Design review of the part built by this model. Coordinates are the model's own, in mm. A direction names the side the tool comes from. Give positions to 0.01 mm unless a question says otherwise; leave off trailing zeros. Order: outer loops, then holes, each group sorted by start corner. A loop starts at its lowest first (then second) coordinate and runs counter-clockwise, first axis right, second up. Notation, with made-up numbers: (86, -1.75) -> (129, -1.75) arc R20 cw to (129, 2.25) -> close; hole circle Ø10 at (40.25, 52.5). An arc over 180 degrees is marked (long way). Use a Markdown table: item, result. Add a question column.
```python
from build123d import *

# Parameters (mm, degrees)
BASE_BLOCK_DEPTH         = 50
POCKET_PROFILE_W         = 20
POCKET_PROFILE_H         = 35
RECTANGULAR_POCKET_DEPTH = 40
SLOT_PROFILE_W           = 30
SLOT_PROFILE_H           = 5
RECTANGULAR_SLOT_DEPTH   = 87.890735985


with BuildPart() as part:
    # Base Block Profile → Base Block (new body)
    with BuildSketch(Plane.XY):
        Polygon((0, 0), (80, 0), (80, 25), (100, 25), (100, 45), (55, 45), (55, 35), (0, 35), align=None)
    extrude(amount=BASE_BLOCK_DEPTH)

    # Pocket Profile → Rectangular Pocket (cut)
    with BuildSketch(Plane.ZY):
        with Locations((25, 17.5)):
            Rectangle(POCKET_PROFILE_W, POCKET_PROFILE_H)
    extrude(amount=-RECTANGULAR_POCKET_DEPTH, mode=Mode.SUBTRACT)

    # Slot Profile → Rectangular Slot (cut, through all)
    with BuildSketch(Plane.ZY.offset(-55)):
        with Locations((25, 42.5)):
            Rectangle(SLOT_PROFILE_W, SLOT_PROFILE_H)
    extrude(amount=-RECTANGULAR_SLOT_DEPTH, mode=Mode.SUBTRACT)


solid = part.part
```
1) Add section D-D (y = 33.5). Give the boundary of the cut face in (x, z).
2) The part is to be moulded in two halves that separate along Z. For faces 1 (the flat face through (55, 39, 25)), 2 (the flat face through (49, 23, 50)), 3 (the flat face through (20, 17, 15)), 4 (the flat face through (77, 42, 10)), say which applies: +Z half, -Z half, draft (parallel to the pull), parting line (faces both ways), or undercut.
3) Add section B-B (y = 41). Give the boundary of the cut face in (x, z), then the cut area to 3 significant figures.
4) Add section C-C (x = 77.5). Give the boundary of the cut face in (y, z).
5) For L1, parallel to Z at x = 89, y = 41; L2, parallel to Z at x = 9, y = 33.5; L3, parallel to X at y = 15, z = 46, list the stretches that pass through material, from the lowest coordinate up. Write a range as [from, to].
6) Machinability: for faces 5 (the flat face through (90, 25, 25)), 6 (the flat face through (28, 35, 36)), 7 (the flat face through (20, 17, 35)), which of the approach directions +Z, -Z, +X, -X, +Y, -Y give a long, thin tool a straight path to every point of the face, cutting with its end or side? Answer none if there is none.
7) Add section A-A (x = 11.5). Give the boundary of the cut face in (y, z), then the cut area to 3 significant figures.
8) Insertion check: pin 1 (12.5 mm diameter, centred on y = 13.5, z = 24, fed in from +X); pin 2 (2 mm diameter, centred on x = 46.5, z = 32, fed in from +Y); pin 3 (6 mm diameter, centred on x = 86.5, z = 29.5, fed in from -Y). Each pin has a flat end and moves straight along its axis. Give the tip position at first contact, or say it passes through.
Worked answers:
| question | item | result |
|---|---|---|
| 1 | outline | (0, 0) -> (100, 0) -> (100, 50) -> (0, 50) -> (0, 35) -> (40, 35) -> (40, 15) -> (0, 15) -> close |
| 2 | face 1 | draft |
| 2 | face 2 | +Z half |
| 2 | face 3 | undercut |
| 2 | face 4 | undercut |
| 3 | outline | (55, 0) -> (100, 0) -> (100, 10) -> (55, 10) -> close; (55, 40) -> (100, 40) -> (100, 50) -> (55, 50) -> close |
| 3 | area | 900 mm^2 |
| 4 | outline | (0, 0) -> (45, 0) -> (45, 10) -> (40, 10) -> (40, 40) -> (45, 40) -> (45, 50) -> (0, 50) -> close |
| 5 | L1 | [0, 10], [40, 50] |
| 5 | L2 | [0, 15], [35, 50] |
| 5 | L3 | [0, 80] |
| 6 | face 5 | +Z, -Z, +X, -Y |
| 6 | face 6 | +Z, -Z, -X, +Y |
| 6 | face 7 | -X, +Y, -Y |
| 7 | outline | (0, 0) -> (35, 0) -> (35, 15) -> (0, 15) -> close; (0, 35) -> (35, 35) -> (35, 50) -> (0, 50) -> close |
| 7 | area | 1,050 mm^2 |
| 8 | pin 1 | x = 80 |
| 8 | pin 2 | y = 35 |
| 8 | pin 3 | y = 25 |
